Read the model definition and answer for the solid it produces. Units are mm, in the model's axes. Face numbers are marked on the shaded views. Coordinates: 2 decimals unless noted, no trailing zeros. Loops run counter-clockwise (first coordinate to the right, second up) from the corner with the lowest first, then second, coordinate; pieces in that order, holes last. Notation, with made-up numbers: M -28,-17 L 25,-17 A14 ccw 25,0 Z; hole C 13,-34.5 d11. An arc over 180 degrees is marked long. Put each result on its own line as item: value.
from build123d import *

# Parameters (mm, degrees)
SKETCH_1_W      = 25
SKETCH_1_H      = 150
SKETCH_1_R      = 6.5
EXTRUDE_1_DEPTH = 8


with BuildPart() as part:
    # 草图1 → 凸台-拉伸1 (new body)
    with BuildSketch(Plane.XY):
        Rectangle(SKETCH_1_W, SKETCH_1_H)
        with Locations((-0.153888597, 54.999784711)):
            Circle(SKETCH_1_R, mode=Mode.SUBTRACT)
        Circle(SKETCH_1_R, mode=Mode.SUBTRACT)
        with Locations((0, -55)):
            Circle(SKETCH_1_R, mode=Mode.SUBTRACT)
    extrude(amount=EXTRUDE_1_DEPTH)


solid = part.part
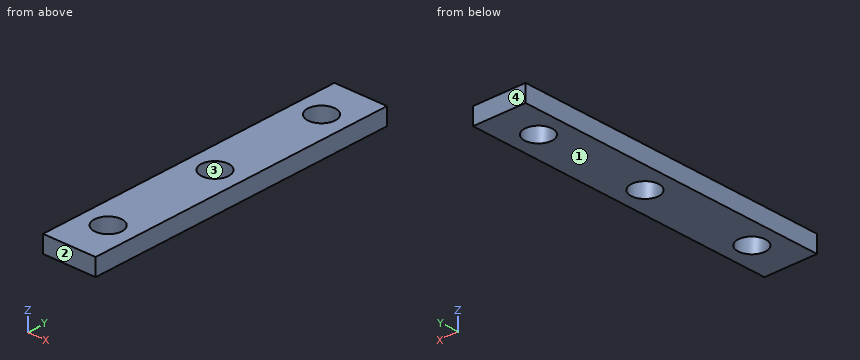
1) Find section D-D, the plane y = 60. Write down the section's boundary in (x, z).
Answer list:
outline: M -12.5,0 L -4.31,0 L -4.31,8 L -12.5,8 Z; M 4,0 L 12.5,0 L 12.5,8 L 4,8 Z
2) Find section B-B, the plane x = -2. Write down the section's boundary in (y, z), plus the area to 3 significant figures.
Answer list:
outline: M -75,0 L -61.18,0 L -61.18,8 L -75,8 Z; M -48.82,0 L -6.18,0 L -6.18,8 L -48.82,8 Z; M 6.18,0 L 48.77,0 L 48.77,8 L 6.18,8 Z; M 61.23,0 L 75,0 L 75,8 L 61.23,8 Z
area: 902 mm^2
3) Straight lines are drawn through the part: line 1 (Y direction, x = 0, z = 5.5); line 2 (Y direction, x = 5.75, z = 4.5); line 3 (X direction, y = -5.5, z = 3). For each, find the intervals that lie inside material, in ascending order. Write a range as [from, to].
Answer list:
line 1: y = [-75, -61.5], [-48.5, -6.5], [6.5, 48.5], [61.5, 75]
line 2: y = [-75, -58.03], [-51.97, -3.03], [3.03, 52.28], [57.72, 75]
line 3: x = [-12.5, -3.46], [3.46, 12.5]
4) Given pin 1 Ø5 at (x, y) = (4.5, -44) entering from -Z, flat-ended and moving along its own axis, determine where the tip first touches the part or whether it passes through.
Answer list:
pin 1: stops at z = 0
5) Find section A-A, the plane y = -55. Write down the section's boundary in (x, z), plus the area to 3 significant figures.
Answer list:
outline: M -12.5,0 L -6.5,0 L -6.5,8 L -12.5,8 Z; M 6.5,0 L 12.5,0 L 12.5,8 L 6.5,8 Z
area: 96.0 mm^2
6) Find section C-C, the plane z = 1.5. Write down the section's boundary in (x, y).
Answer list:
outline: M -12.5,-75 L 12.5,-75 L 12.5,75 L -12.5,75 Z; hole C -0.15,55 d13; hole C 0,-55 d13; hole C 0,0 d13
7) Determine the mould class of the marked faces 1, 2, 3 and 4 for opening direction Y: released by +Y, released by -Y, zero draft, split by the parting line, or undercut.
Answer list:
face 1: zero draft
face 2: released by -Y
face 3: undercut
face 4: released by +Y
